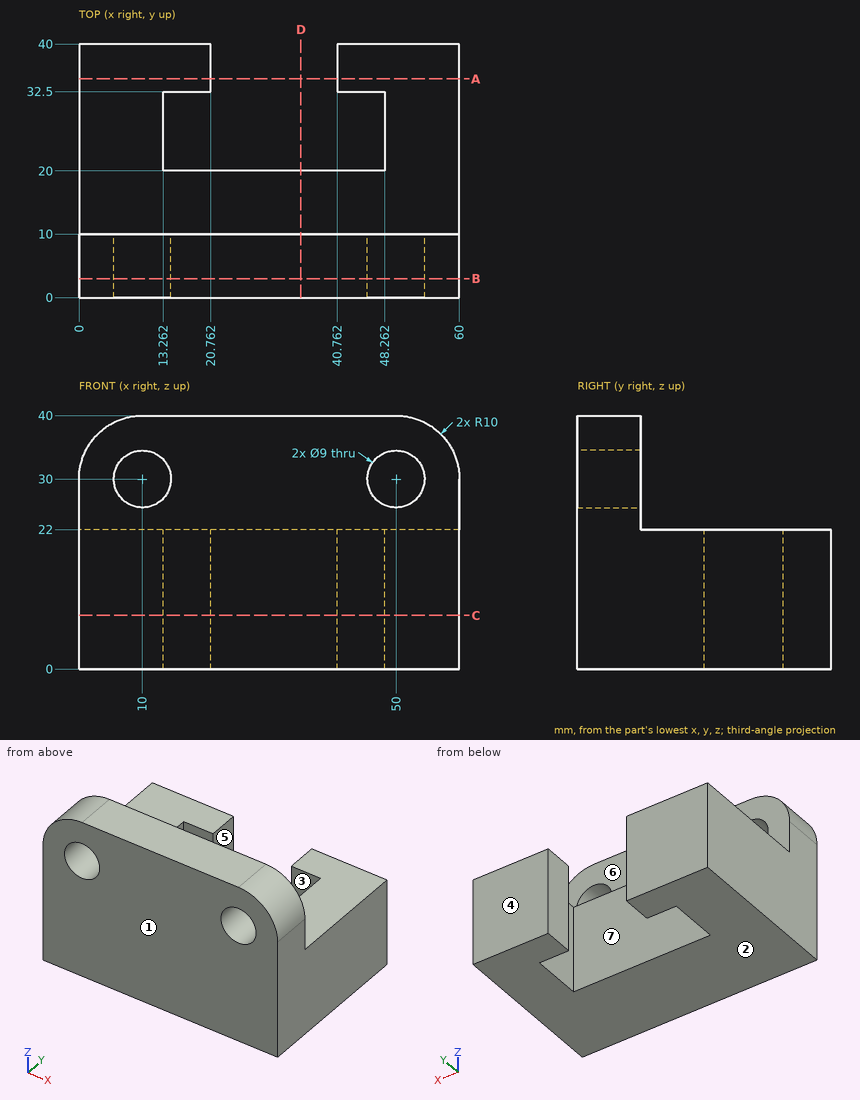
Geometry check sheet. Reference: drawing and pictorial views, mm from the part's lowest x, y, z. A direction names the side the tool comes from. Round coordinates to 2 decimals unless told otherwise and drop trailing zeros. Loops run counter-clockwise (first coordinate to the right, second up) from the corner with the lowest first, then second, coordinate; pieces in that order, holes last. Notation, with made-up numbers: (72.25, 61) -> (80.25, 61) arc R27 ccw to (80.25, 88) -> close; hole circle Ø3 at (-24, 14.25). An arc over 180 degrees is marked (long way). Use a Markdown table: item, result.
(1) Sectioned sample at A-A (y = 34.5). Enter the section's corners in (x, z).
Calculated:
| item | result |
|---|---|
| outline | (0, 0) -> (20.76, 0) -> (20.76, 22) -> (0, 22) -> close; (40.76, 0) -> (60, 0) -> (60, 22) -> (40.76, 22) -> close |
(2) Sectioned sample at B-B (y = 3). Enter the section's corners in (x, z), then the cut area to 3 significant figures.
Calculated:
| item | result |
|---|---|
| outline | (0, 0) -> (60, 0) -> (60, 30) arc R10 ccw to (50, 40) -> (10, 40) arc R10 ccw to (0, 30) -> close; hole circle Ø9 at (10, 30); hole circle Ø9 at (50, 30) |
| area | 2,230 mm² |
(3) Sectioned sample at D-D (x = 35). Enter the section's corners in (y, z).
Calculated:
| item | result |
|---|---|
| outline | (0, 0) -> (20, 0) -> (20, 22) -> (10, 22) -> (10, 40) -> (0, 40) -> close |
(4) Go/stop test with flat-tipped pins: P1, Ø5.5, axis at x = 41.5, z = 27, coming from the +Y side; P2, Ø12, axis at x = 50, y = 24, coming from the +Z side; P3, Ø10, axis at x = 27.5, z = 13, coming from the +Y side. Record where each tip stops, or that it passes through.
Calculated:
| item | result |
|---|---|
| P1 | y = 10 |
| P2 | z = 22 |
| P3 | y = 20 |
(5) Set-up check for the marked faces 4, 5, 6 and 7: record each of +Z, -Z, +X, -X, +Y, -Y from which the full face is reachable in a straight line by a thin tool's end or side.
Calculated:
| item | result |
|---|---|
| face 4 | +Z, -Z, +X, -X, +Y |
| face 5 | +Z, -Z, +Y |
| face 6 | +Z, +X, -X, +Y |
| face 7 | +Z, -Z |
(6) Sectioned sample at C-C (z = 8.5). Enter the section's corners in (x, y).
Calculated:
| item | result |
|---|---|
| outline | (0, 0) -> (60, 0) -> (60, 40) -> (40.76, 40) -> (40.76, 32.5) -> (48.26, 32.5) -> (48.26, 20) -> (13.26, 20) -> (13.26, 32.5) -> (20.76, 32.5) -> (20.76, 40) -> (0, 40) -> close |
(7) Mould release check, pull along Y, two halves, no side actions. Record for the marked faces 1, 2 and 3: released by +Y, released by -Y, zero draft, split by the parting line, or undercut.
Calculated:
| item | result |
|---|---|
| face 1 | released by -Y |
| face 2 | zero draft |
| face 3 | undercut |
(8) Scan lines: probe 1 along X at (y, z) = (6, 30); probe 2 along X at (y, z) = (21.5, 6.5); probe 3 along Y at (x, z) = (22.5, 33). Record each from-to range of solid material in increasing order.
Calculated:
| item | result |
|---|---|
| probe 1 | 0 to 5.5, 14.5 to 45.5, 54.5 to 60 |
| probe 2 | 0 to 13.26, 48.26 to 60 |
| probe 3 | 0 to 10 |
